The model under review builds one solid part; all positions refer to its coordinate system, in mm. A direction names the side the tool comes from. Round coordinates to 2 decimals unless told otherwise and drop trailing zeros. Write each loop counter-clockwise with the first axis right and the second up, starting at its lowest first coordinate (ties: lowest second). Pieces come first, ordered by that corner, then holes. Notation, with made-up numbers: (40, 53.25) - (89, 53.25) arc R27 cw to (89, 87.25) - close; hole circle Ø6 at (29, 37.5). An arc over 180 degrees is marked (long way). Write each question's results on one line, items separated by ' | '.
```python
from build123d import *

# Parameters (mm, degrees)
SKETCH1_R               = 16
BOSS_EXTRUDE1_DEPTH     = 175
SKETCH2_R               = 18.5
BOSS_EXTRUDE2_DEPTH     = 5
SKETCH3_R               = 10
CUT_EXTRUDE1_DEPTH      = 100
SKETCH4_R               = 6
CUT_EXTRUDE2_DEPTH      = 8000
CUT_EXTRUDE3_DEPTH      = 182.891451146
CUT_EXTRUDE3_DEPTH_BACK = 182.891451146


with BuildPart() as part:
    # Sketch1 → Boss-Extrude1 (new body)
    with BuildSketch(Plane(origin=(0, 0, 0), x_dir=(0, 0, -1), z_dir=(1, 0, 0))):
        Circle(SKETCH1_R)
    extrude(amount=BOSS_EXTRUDE1_DEPTH)

    # Sketch2 → Boss-Extrude2 (add)
    with BuildSketch(Plane(origin=(175, 0, 0), x_dir=(0, 0, -1), z_dir=(1, 0, 0))):
        Circle(SKETCH2_R)
    extrude(amount=BOSS_EXTRUDE2_DEPTH)

    # Sketch3 → Cut-Extrude1 (cut)
    with BuildSketch(Plane(origin=(180, 0, 0), x_dir=(0, 0, -1), z_dir=(1, 0, 0))):
        Circle(SKETCH3_R)
    extrude(amount=-CUT_EXTRUDE1_DEPTH, mode=Mode.SUBTRACT)

    # Sketch4 → Cut-Extrude2 (cut)
    with BuildSketch(Plane(origin=(180, 0, 0), x_dir=(0, 0, -1), z_dir=(1, 0, 0))):
        Circle(SKETCH4_R)
    extrude(amount=-CUT_EXTRUDE2_DEPTH, mode=Mode.SUBTRACT)

    # Sketch5 → Cut-Revolve1 (revolve, cut)
    with BuildSketch(Plane.XY, mode=Mode.PRIVATE) as cut_revolve1_sk:
        Polygon((0, 0), (50, 0), (50, 6), (0, 11), align=None)
    revolve(cut_revolve1_sk.sketch.rotate(Axis((0, 0, 0), (1, 0, 0)), 270), axis=Axis((0, 0, 0), (1, 0, 0)), mode=Mode.SUBTRACT)

    # Sketch6 → Cut-Extrude3 (cut, two sides: drawn at the far end of the back side and taken through both)
    with BuildSketch(Plane.XY.offset(-CUT_EXTRUDE3_DEPTH_BACK)):
        Polygon((69.995219392, 16.697170081), (66.404780608, 16.697170081), (67.635, 13.317170081), (68.765, 13.317170081), align=None)
        Polygon((72.345, 13.317170081), (73.475, 13.317170081), (74.705219392, 16.697170081), (71.114780608, 16.697170081), align=None)
        Polygon((77.055, 13.317170081), (78.185, 13.317170081), (79.415219392, 16.697170081), (75.824780608, 16.697170081), align=None)
        Polygon((81.765, 13.317170081), (82.895, 13.317170081), (84.125219392, 16.697170081), (80.534780608, 16.697170081), align=None)
        Polygon((86.475, 13.317170081), (87.605, 13.317170081), (88.835219392, 16.697170081), (85.244780608, 16.697170081), align=None)
        Polygon((91.185, 13.317170081), (92.315, 13.317170081), (93.545219392, 16.697170081), (89.954780608, 16.697170081), align=None)
        Polygon((95.895, 13.317170081), (97.025, 13.317170081), (98.255219392, 16.697170081), (94.664780608, 16.697170081), align=None)
        Polygon((100.605, 13.317170081), (101.735, 13.317170081), (102.965219392, 16.697170081), (99.374780608, 16.697170081), align=None)
        Polygon((105.315, 13.317170081), (106.445, 13.317170081), (107.675219392, 16.697170081), (104.084780608, 16.697170081), align=None)
        Polygon((110.025, 13.317170081), (111.155, 13.317170081), (112.385219392, 16.697170081), (108.794780608, 16.697170081), align=None)
        Polygon((114.735, 13.317170081), (115.865, 13.317170081), (117.095219392, 16.697170081), (113.504780608, 16.697170081), align=None)
        Polygon((119.445, 13.317170081), (120.575, 13.317170081), (121.805219392, 16.697170081), (118.214780608, 16.697170081), align=None)
        Polygon((124.155, 13.317170081), (125.285, 13.317170081), (126.515219392, 16.697170081), (122.924780608, 16.697170081), align=None)
        Polygon((128.865, 13.317170081), (129.995, 13.317170081), (131.225219392, 16.697170081), (127.634780608, 16.697170081), align=None)
    extrude(amount=CUT_EXTRUDE3_DEPTH + CUT_EXTRUDE3_DEPTH_BACK, mode=Mode.SUBTRACT)


solid = part.part
```
Q1. Insertion check: P1, Ø10, axis at x = 156, y = 11, coming from the +Z side; P2, Ø3, axis at x = 75, y = 6.5, coming from the +Z side; P3, Ø10, axis at x = 149.5, z = -8.5, coming from the -Y side. Each pin has a flat end and moves straight along its axis. Give the tip position at first contact, or say it passes through.
Evaluation:
P1: stops at z = 14.83 | P2: stops at z = 15.2 | P3: stops at y = -15.61
Q2. We need section A-A (y = 0). State the section outline as (x, z) points, plus the area to 4 significant figures.
Evaluation:
outline: (0, -16) - (175, -16) - (175, -18.5) - (180, -18.5) - (180, -10) - (80, -10) - (80, -6) - (50, -6) - (0, -11) - close; (0, 11) - (50, 6) - (80, 6) - (80, 10) - (180, 10) - (180, 18.5) - (175, 18.5) - (175, 16) - (0, 16) - close | area: 2,575 mm^2
Q3. The part is to be moulded in two halves that separate along Y. For faces 1 (the cylindrical face through (65, 0, 6)), 2 (the cylindrical face through (86.28, -15.62, 3.47)), 3 (the flat face through (180, -8, -8)), say which applies: released by +Y, released by -Y, zero draft, split by the parting line, or undercut.
Evaluation:
face 1: undercut | face 2: split by the parting line | face 3: zero draft
Q4. Tool access review of faces 4 (the flat face through (175, 15, 6)), 5 (the cylindrical face through (130.7, -9.76, 2.17)), 6 (the flat face through (0, 11, -3)): name each direction out of +Z, -Z, +X, -X, +Y, -Y from which nothing blocks a thin tool from reaching the whole face with its end or side.
Evaluation:
face 4: -X | face 5: +X | face 6: +Z, -Z, -X, +Y, -Y
Q5. For probe 1 along Y at (x, z) = (56, 0); probe 2 along Y at (x, z) = (160, 0); probe 3 along Y at (x, z) = (163.5, -12.5), list the stretches that pass through material, from the lowest coordinate up.
Evaluation:
probe 1: y = -16 to -6, 6 to 16 | probe 2: y = -16 to -10, 10 to 16 | probe 3: y = -9.99 to 9.99
Q6. We need section B-B (x = 139). State the section outline as (y, z) points, plus the area to 3 significant figures.
Evaluation:
outline: circle Ø32 at (0, 0); hole circle Ø20 at (0, 0) | area: 490 mm^2
Q7. We need section C-C (z = 13.5). State the section outline as (x, y) points, plus the area to 3 significant figures.
Evaluation:
outline: (0, -8.59) - (175, -8.59) - (175, -12.65) - (180, -12.65) - (180, 12.65) - (175, 12.65) - (175, 8.59) - (0, 8.59) - close | area: 3,130 mm^2
